Could you check a few things on this model? Use its own coordinates, in mm. Face numbers are marked on the shaded views. Coordinates: 2 decimals unless noted, no trailing zeros. Order: outer loops, then holes, each group sorted by start corner. A loop starts at its lowest first (then second) coordinate and runs counter-clockwise, first axis right, second up. Notation, with made-up numbers: (36.25, 6) -> (92.25, 6) arc R13 ccw to (92.25, 15) -> close; hole circle Ø10 at (13.25, 20). An arc over 180 degrees is marked (long way). Put each result on its own line as item: value. Start each with the question number.
Q1. If we section it at B-B (y = 3.4): Please give me the cut outline in (x, z).
Q2. If we section it at D-D (z = 18.5): Please give me the cut outline in (x, y).
Q3. Please list where these lines run through material, in increasing order: line 1 along X through (y, z) = (1.1, 85); line 2 along Z through (x, y) = (5, 3.5); line 3 along Z through (x, y) = (5.5, 3.55).
Q4. We'd pull the mould along Y, two halves only. Please class the marked faces 1 and 2: +Y half, -Y half, draft (parallel to the pull), parting line (faces both ways), or undercut.
Q5. If we section it at A-A (z = 0): Please give me the cut outline in (x, y).
Q6. Will these pins go through, and if not, where does the flat tip stop? pin 1 (4.5 mm diameter, centred on x = 54, z = 85, fed in from +Y); pin 2 (2 mm diameter, centred on y = 3, z = 7, fed in from +X).
Q7. If we section it at C-C (x = -6.5): Please give me the cut outline in (y, z), and give its area (3 significant figures).
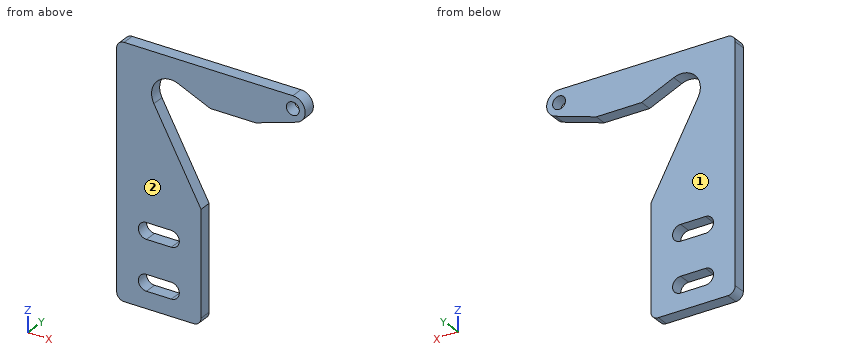
from build123d import *

# Parameters (mm, degrees)
SKETCH1_R           = 2.6
BOSS_EXTRUDE1_DEPTH = 5
FILLET1_R           = 3


with BuildPart() as part:
    # Sketch1 → Boss-Extrude1 (new body)
    with BuildSketch(Plane(origin=(0, 0, 0), x_dir=(1, 0, 0), z_dir=(0, 1, 0))):
        with BuildLine():
            Line((-17, 10), (-17, -90))
            Line((-17, -90), (54, -90))
            ThreePointArc((54, -90), (58.941222292, -85.764409749), (55.510847396, -80.233728906))
            Line((55.510847396, -80.233728906), (39, -75))
            Line((39, -75), (20.726086957, -75))
            Line((20.726086957, -75), (7.79590612, -80.661902004))
            ThreePointArc((7.79590612, -80.661902004), (-0.909612834, -78.829253465), (-2, -70))
            Line((-2, -70), (17, -35))
            Line((17, -35), (17, 10))
            Line((17, 10), (-17, 10))
        make_face()
        with Locations(Location((54, -85, 0), (0, 0, 270))):
            Circle(SKETCH1_R, mode=Mode.SUBTRACT)
        with BuildLine():
            Line((5, -3.25), (-5, -3.25))
            ThreePointArc((-5, -3.25), (-8.25, 0), (-5, 3.25))
            Line((-5, 3.25), (5, 3.25))
            ThreePointArc((5, 3.25), (8.25, 0), (5, -3.25))
        make_face(mode=Mode.SUBTRACT)
        with BuildLine():
            Line((5, -23.25), (-5, -23.25))
            ThreePointArc((-5, -23.25), (-8.25, -20), (-5, -16.75))
            Line((-5, -16.75), (5, -16.75))
            ThreePointArc((5, -16.75), (8.25, -20), (5, -23.25))
        make_face(mode=Mode.SUBTRACT)
    extrude(amount=BOSS_EXTRUDE1_DEPTH)

    # Fillet1
    fillet1_edges = [part.edges().sort_by_distance(p)[0] for p in [
        (17, 2.5, -10),
        (-17, 2.5, 90),
        (-17, 2.5, -10),
    ]]
    fillet(fillet1_edges, radius=FILLET1_R)


solid = part.part
The answers:
1. outline: (-17, -7) arc R3 ccw to (-14, -10) -> (14, -10) arc R3 ccw to (17, -7) -> (17, 35) -> (-2, 70) arc R7.65 cw to (7.8, 80.66) -> (20.73, 75) -> (39, 75) -> (55.51, 80.23) arc R5 ccw to (54, 90) -> (-14, 90) arc R3 ccw to (-17, 87) -> close; hole (-5, -3.25) -> (5, -3.25) arc R3.25 ccw to (5, 3.25) -> (-5, 3.25) arc R3.25 ccw to start; hole (-5, 16.75) -> (5, 16.75) arc R3.25 ccw to (5, 23.25) -> (-5, 23.25) arc R3.25 ccw to start; hole circle Ø5.2 at (54, 85)
2. outline: (-17, 0) -> (-7.88, 0) -> (-7.88, 5) -> (-17, 5) -> close; (7.88, 0) -> (17, 0) -> (17, 5) -> (7.88, 5) -> close
3. line 1: -17 to 51.4, 56.6 to 59
3. line 2: -10 to -3.25, 3.25 to 16.75, 23.25 to 57.11, 81.3 to 90
3. line 3: -10 to -3.21, 3.21 to 16.79, 23.21 to 56.18, 81.27 to 90
4. face 1: +Y half
4. face 2: -Y half
5. outline: (-17, 0) -> (-8.25, 0) -> (-8.25, 5) -> (-17, 5) -> close; (8.25, 0) -> (17, 0) -> (17, 5) -> (8.25, 5) -> close
6. pin 1: through
6. pin 2: x = 17
7. outline: (0, -10) -> (5, -10) -> (5, -2.88) -> (0, -2.88) -> close; (0, 2.88) -> (5, 2.88) -> (5, 17.12) -> (0, 17.12) -> close; (0, 22.88) -> (5, 22.88) -> (5, 90) -> (0, 90) -> close
7. area: 442 mm^2
